Print and shaded views of the part. All mm, measured from the part's lowest x, y and z. A direction names the side the tool comes from. Round coordinates to 2 decimals unless told otherwise and drop trailing zeros. Write each loop counter-clockwise with the first axis right and the second up, starting at its lowest first coordinate (ties: lowest second). Pieces come first, ordered by that corner, then holes. Notation, with made-up numbers: (-20.5, 56.5) -> (-13.5, 56.5) arc R30 cw to (-13.5, 87.5) -> close; hole circle Ø4 at (80.5, 34.5). An arc over 180 degrees is marked (long way). Return JSON: item names as keys, results as strings. Group by question number.
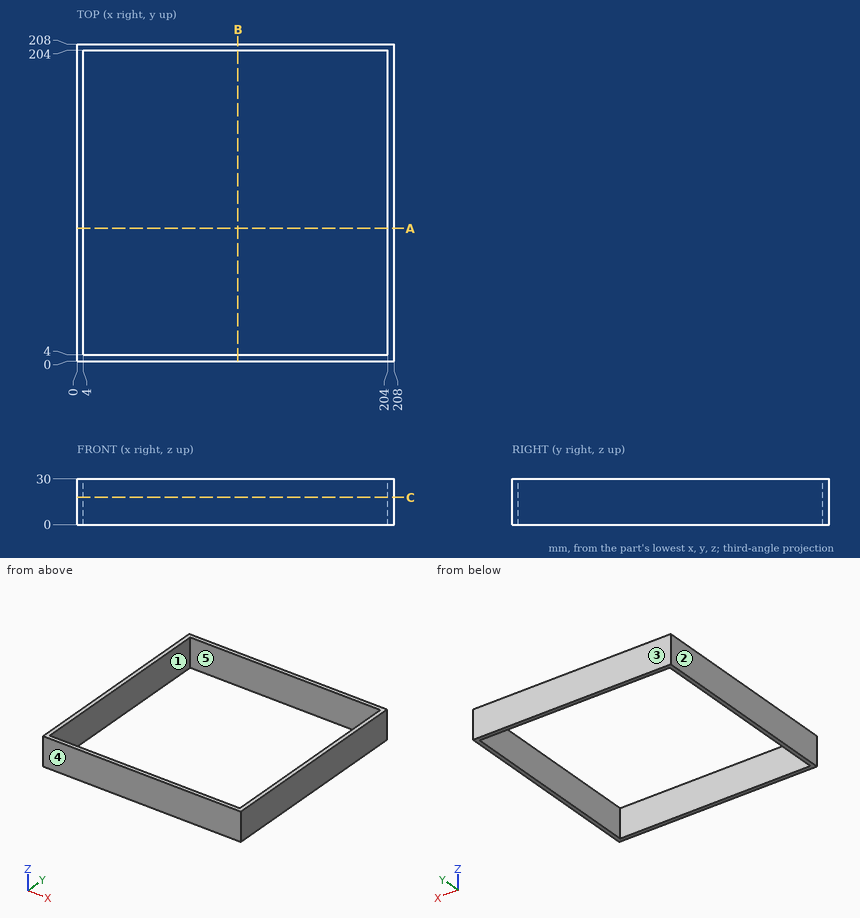
Item 1: Cut at C-C (z = 18). Write the cut outline in (x, y), then the cut area to 3 significant figures.
Item 2: Cut at A-A (y = 87). Write the cut outline in (x, z).
Item 3: Which spindle directions (+Z, -Z, +X, -X, +Y, -Y) get a long thin tool onto all of the face, cutting with end or side? Do the marked faces 4 and 5. Say none if no direction does.
Item 4: Wall check: L1, parallel to Y at x = 105, z = 22.25. Give the ranges that are in metal, low to high.
Item 5: Two-plate mould, pull along Y, no slides. Class the marked faces 1, 2 and 3: released by +Y, released by -Y, zero draft, split by the parting line, or undercut.
Checks:
{
 "1": {"outline": "(0, 0) -> (208, 0) -> (208, 208) -> (0, 208) -> close; hole (4, 4) -> (204, 4) -> (204, 204) -> (4, 204) -> close", "area": "3,260 mm2"},
 "2": {"outline": "(0, 0) -> (4, 0) -> (4, 30) -> (0, 30) -> close; (204, 0) -> (208, 0) -> (208, 30) -> (204, 30) -> close"},
 "3": {"face 4": "+Z, -Z, +X, -X, -Y", "face 5": "+Z, -Z"},
 "4": {"L1": "y = 0 to 4, 204 to 208"},
 "5": {"face 1": "undercut", "face 2": "zero draft", "face 3": "released by +Y"}
}
